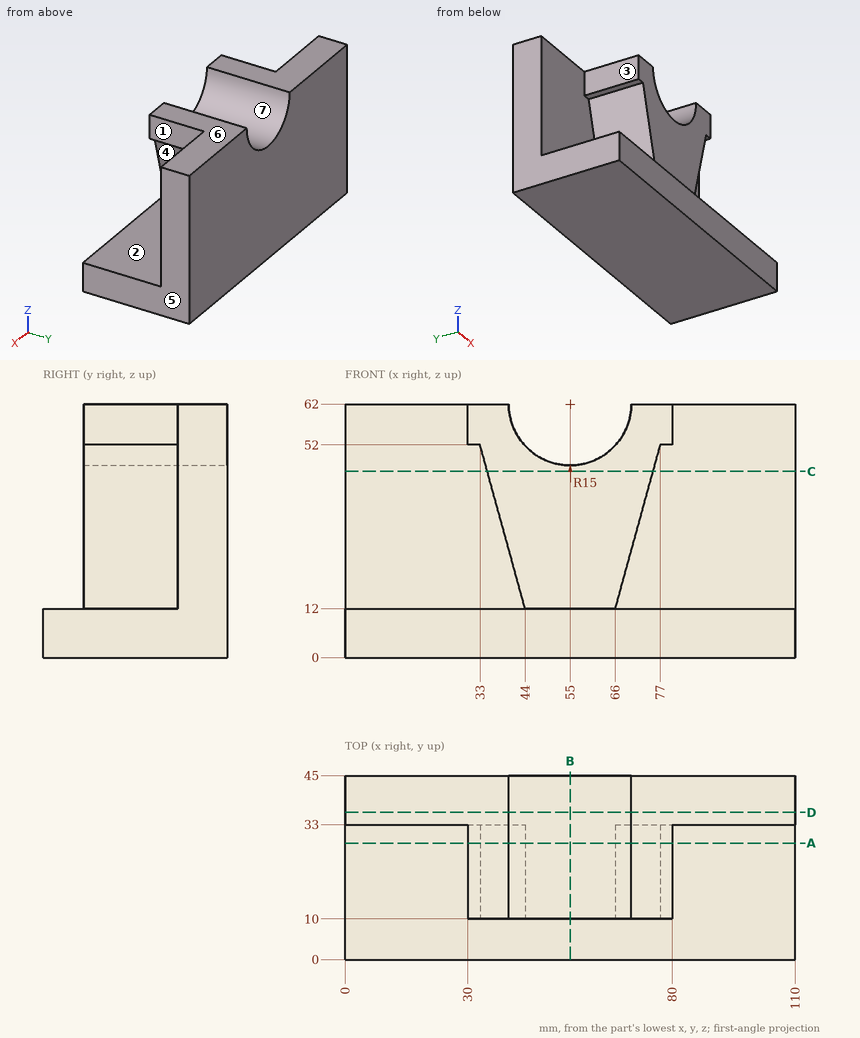
Study the drawing (mm; zero at the part's minimum x, y, z) and answer. A direction names the side the tool comes from. Coordinates: 2 decimals unless noted, no trailing zeros. Write each loop counter-clockwise with the first axis right and the second up, starting at its lowest first coordinate (ties: lowest second). Pieces come first, ordered by that corner, then holes. Notation, with made-up numbers: (26, 83.25) - (72, 83.25) arc R18 ccw to (72, 102.25) - close; hole circle Ø8 at (-29, -13). An arc over 180 degrees is marked (long way). Put each result on its own line as item: value.
1. Find the intervals of material crossed by line 1 along Y through (x, z) = (101.5, 27); line 2 along Z through (x, y) = (92, 5.5); line 3 along Y through (x, z) = (61, 20), in increasing order. Write a range as from..to.
Answer sheet:
line 1: y = 33..45
line 2: z = 0..12
line 3: y = 10..45
2. Determine the mould class of the marked faces 5, 6 and 7 for opening direction X: pulls with the +X half, pulls with the -X half, needs draft (parallel to the pull), parting line crosses it, or undercut.
Answer sheet:
face 5: pulls with the +X half
face 6: needs draft
face 7: undercut
3. The part is cut by section D-D on y = 36. Give the vertices of the cut face in (x, z).
Answer sheet:
outline: (0, 0) - (110, 0) - (110, 62) - (70, 62) arc R15 cw to (40, 62) - (0, 62) - close
4. A tool of negligible diameter and unlimited length cuts with its end or side. For the marked faces 1, 2, 3 and 4, from which of +Z, -Z, +X, -X, +Y, -Y can it reach the whole face along a straight path? Write none if from no direction.
Answer sheet:
face 1: +Z, +X, -Y
face 2: -Y
face 3: +Z, -X, -Y
face 4: +X, -Y
5. The part is cut by section A-A on y = 28.5. Give the vertices of the cut face in (x, z).
Answer sheet:
outline: (0, 0) - (110, 0) - (110, 12) - (66, 12) - (77, 52) - (80, 52) - (80, 62) - (70, 62) arc R15 cw to (40, 62) - (30, 62) - (30, 52) - (33, 52) - (44, 12) - (0, 12) - close
6. The part is cut by section B-B on x = 55. Give the vertices of the cut face in (y, z), plus the area to 4 significant figures.
Answer sheet:
outline: (0, 0) - (45, 0) - (45, 47) - (10, 47) - (10, 12) - (0, 12) - close
area: 1,765 mm^2
7. Flat-ended cylindrical pins translate along their axes: pin 1 Ø2 at (x, z) = (32.5, 25) entering from -Y; pin 2 Ø15 at (x, z) = (56.5, 40.5) entering from -Y; pin 3 Ø11 at (y, z) = (25.5, 59) entering from -X. Find the tip coordinate at first contact, or state that the pin passes through.
Answer sheet:
pin 1: stops at y = 33
pin 2: stops at y = 10
pin 3: stops at x = 30
8. The part is cut by section C-C on z = 45.5. Give the vertices of the cut face in (x, y), plus the area to 3 significant figures.
Answer sheet:
outline: (0, 33) - (34.79, 33) - (34.79, 10) - (75.21, 10) - (75.21, 33) - (110, 33) - (110, 45) - (0, 45) - close
area: 2,250 mm^2
